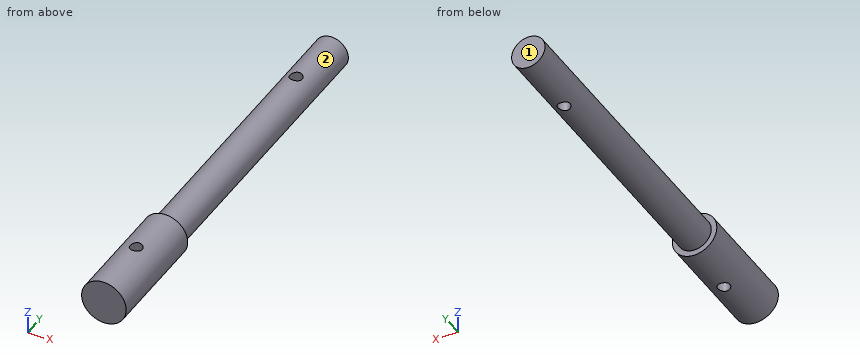
from build123d import *

# Parameters (mm, degrees)
SKETCH_2_R          = 1.1
CUT_EXTRUDE_1_DEPTH = 15


with BuildPart() as part:
    # 草图1 → 旋转1 (revolve)
    with BuildSketch(Plane.XY, mode=Mode.PRIVATE) as revolve_1_sk:
        Polygon((0, 68.097402597), (3, 68.097402597), (3, 14.097402597), (4, 14.097402597), (4, -5.902597403), (0, -5.902597403), align=None)
    revolve(revolve_1_sk.sketch.rotate(Axis((0, 0, 0), (0, 1, 0)), 90), axis=Axis((0, 0, 0), (0, 1, 0)))

    # 草图2 → 切除-拉伸1 (cut, symmetric)
    with BuildSketch(Plane.XY):
        with Locations((0, 56.497402597)):
            Circle(SKETCH_2_R)
        with Locations((0, 4.597402597)):
            Circle(SKETCH_2_R)
    extrude(amount=CUT_EXTRUDE_1_DEPTH, both=True, mode=Mode.SUBTRACT)


solid = part.part
Work out the finished part from the listing and answer in its coordinate system (mm). Face numbers are marked on the shaded views. A direction names the side the tool comes from. Round coordinates to 2 decimals unless told otherwise and drop trailing zeros. Write each loop counter-clockwise with the first axis right and the second up, starting at its lowest first coordinate (ties: lowest second). Pieces come first, ordered by that corner, then holes. Notation, with made-up numbers: (-28, -36) -> (-9, -36) arc R10 cw to (-9, -20) -> close; hole circle Ø1 at (-13.75, 36). An arc over 180 degrees is marked (long way). Answer as CSV lines item,"result". Start each with the question number.
(1) A tool of negligible diameter and unlimited length cuts with its end or side. For the marked faces 1 and 2, from which of +Z, -Z, +X, -X, +Y, -Y can it reach the whole face along a straight path? Write none if from no direction.
(2) Find the intervals of material crossed by probe 1 along Y at (x, z) = (0, -1.5); probe 2 along Y at (x, z) = (0.5, -1.25); probe 3 along Y at (x, z) = (3.5, 1.25), in increasing order.
(3) The part is cut by section A-A, the plane z = -1.25. Give the vertices of the cut face in (x, y), then the cut area to 3 significant figures.
(4) Each of these flat-tipped pins is pushed along its axis until it touches: pin 1 (2.5 mm diameter, centred on x = 0, y = 56.5, fed in from +Z); pin 2 (4 mm diameter, centred on x = -1, y = 23, fed in from -Z); pin 3 (4 mm diameter, centred on y = 58, z = 3, fed in from -X). Where does it stop, or does it pass through?
(5) The part is cut by section B-B, the plane y = 18.5. Give the vertices of the cut face in (x, z), then the cut area to 3 significant figures.
Output values:
1,face 1,"+Z, -Z, +X, -X, +Y"
1,face 2,"+Y"
2,probe 1,"y = -5.9 to 3.5, 5.7 to 55.4, 57.6 to 68.1"
2,probe 2,"y = -5.9 to 3.62, 5.58 to 55.52, 57.48 to 68.1"
2,probe 3,"y = -5.9 to 14.1"
3,outline,"(-3.8, -5.9) -> (3.8, -5.9) -> (3.8, 14.1) -> (2.73, 14.1) -> (2.73, 68.1) -> (-2.73, 68.1) -> (-2.73, 14.1) -> (-3.8, 14.1) -> close; hole circle Ø2.2 at (0, 4.6); hole circle Ø2.2 at (0, 56.5)"
3,area,"439 mm²"
4,pin 1,"stops at z = 3"
4,pin 2,"stops at z = -3"
4,pin 3,"stops at x = -2.83"
5,outline,"circle Ø6 at (0, 0)"
5,area,"28.3 mm²"
